For this review, take the finished solid that the model builds, in its own axes (mm). A direction names the side the tool comes from. Round coordinates to 2 decimals unless told otherwise and drop trailing zeros. One line per item, written item: value. Start each with the question number.
Q1. For probe 1 along Y at (x, z) = (-1.5, 0); probe 2 along Y at (x, z) = (-1.75, 1.5); probe 3 along Y at (x, z) = (-3.7, 0), list the stretches that pass through material, from the lowest coordinate up.
Q2. Tool access review of faces 1 (the face through (-3.393, 1, 1)), 2 (the face through (-1.83, 2.8, -3.65)): name each direction out of +Z, -Z, +X, -X, +Y, -Y from which nothing blocks a thin tool from reaching the whole face with its end or side.
Q3. Mouldability with a two-part tool opening along Z and no side actions: class faces 3 (the face through (-3.91, 2.8, -3.65)), 4 (the face through (0, 0, -1)), 5 (the face through (-2.764, 4.267, 2.22)) as +Z half, -Z half, draft (parallel to the pull), parting line (faces both ways), or undercut.
Q4. Clearance check with flat-ended pins moving along their axes: pin 1 Ø1 at (y, z) = (3, -1.5) entering from -X; pin 2 Ø1.5 at (x, z) = (-1.5, 4) entering from +Y; pin 3 Ø3 at (y, z) = (-3.5, 2.5) entering from +X. State where each tip first meets the part, or that it passes through.
```python
from build123d import *


with BuildPart() as part:
    # Sketch1 → Revolve1 (revolve)
    with BuildSketch(Plane.XY, mode=Mode.PRIVATE) as revolve1_sk:
        Polygon((-4.442951931, 5.01), (-4.442951931, 4.6), (-3.392951931, 4.6), (-3.392951931, 1.248035053), (-4.442951931, 0.813110813), (-4.55, 0), (-2.75, 0), (-2.75, 0.75), (0, 0.75), (0, 1.6), (-0.4, 2), (-1.642951931, 2), (-2.642951931, 3), (-2.642951931, 4.6), (-1.042951931, 4.6), (-1.042951931, 5.01), (-1.242951931, 4.81), (-4.242951931, 4.81), align=None)
    revolve(revolve1_sk.sketch.rotate(Axis((-2.75, 0, 0), (1, 0, 0)), 90), axis=Axis((-2.75, 0, 0), (1, 0, 0)))


solid = part.part
```
Result set:
1. probe 1: y = -4.81 to -4.6, -2 to -0.75, 0.75 to 2, 4.6 to 4.81
1. probe 2: y = -4.57 to -4.35, -1.48 to 1.48, 4.35 to 4.57
1. probe 3: y = -4.81 to -4.6, -1.12 to 1.12, 4.6 to 4.81
2. face 1: -X
2. face 2: +X
3. face 3: undercut
3. face 4: draft
3. face 5: parting line
4. pin 1: stops at x = -3.39
4. pin 2: stops at y = 3.67
4. pin 3: stops at x = -1.04
